For this review, take the finished solid that the model builds, in its own axes (mm). Face numbers are marked on the shaded views. A direction names the side the tool comes from. Coordinates: 2 decimals unless noted, no trailing zeros. Loops run counter-clockwise (first coordinate to the right, second up) from the corner with the lowest first, then second, coordinate; pieces in that order, holes last. Notation, with made-up numbers: (25, -26.5) -> (52, -26.5) arc R7 cw to (52, -19.5) -> close; hole circle Ø9 at (53, -19). An arc over 180 degrees is marked (long way). Use a Markdown table: item, result.
from build123d import *

# Parameters (mm, degrees)
EXTRUDE_1_DEPTH     = 30
SKETCH_3_R          = 9.25
CUT_EXTRUDE_1_DEPTH = 30
SKETCH_4_R          = 2.75
CUT_EXTRUDE_2_DEPTH = 30
CHAMFER_1_SIZE      = 5


with BuildPart() as part:
    # 草图1 → 凸台-拉伸1 (new body)
    with BuildSketch(Plane.XY):
        with BuildLine():
            Line((0, 0), (40, 0))
            ThreePointArc((40, 0), (43.535533906, -1.464466094), (45, -5))
            Line((45, -5), (45, -55))
            Line((45, -55), (41, -55))
            Line((41, -55), (41, -5))
            ThreePointArc((41, -5), (40.707106781, -4.292893219), (40, -4))
            Line((40, -4), (0, -4))
            Line((0, -4), (0, 0))
        make_face()
    extrude(amount=EXTRUDE_1_DEPTH)

    # 草图3 → 切除-拉伸1 (cut)
    with BuildSketch(Plane(origin=(45, 0, 0), x_dir=(0, 0, -1), z_dir=(1, 0, 0))):
        with Locations((-15, -40)):
            Circle(SKETCH_3_R)
    extrude(amount=-CUT_EXTRUDE_1_DEPTH, mode=Mode.SUBTRACT)

    # 草图4 → 切除-拉伸2 (cut)
    with BuildSketch(Plane(origin=(0, 0, 0), x_dir=(1, 0, 0), z_dir=(0, 1, 0))):
        with Locations(Location((5, -5, 0), (0, 0, 180))):
            Circle(SKETCH_4_R)
        with Locations(Location((25, -25, 0), (0, 0, 180))):
            Circle(SKETCH_4_R)
    extrude(amount=-CUT_EXTRUDE_2_DEPTH, mode=Mode.SUBTRACT)

    # 倒角1
    chamfer_1_edges = [part.edges().sort_by_distance(p)[0] for p in [
        (43, -55, 0),
        (0, -2, 30),
        (43, -55, 30),
        (0, -2, 0),
    ]]
    chamfer(chamfer_1_edges, length=CHAMFER_1_SIZE)


solid = part.part
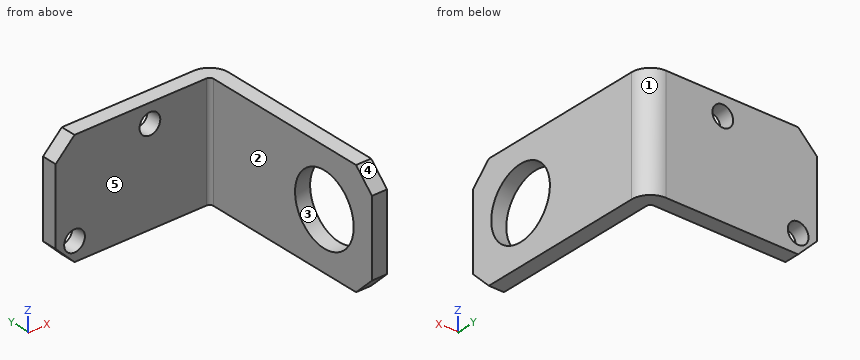
(1) Mouldability with a two-part tool opening along Y and no side actions: class the marked faces 1, 2 and 3 as pulls with the +Y half, pulls with the -Y half, needs draft (parallel to the pull), parting line crosses it, or undercut.
Found:
| item | result |
|---|---|
| face 1 | pulls with the +Y half |
| face 2 | needs draft |
| face 3 | undercut |
(2) Take a section at D-D on z = 25.75. Write out the cut boundary in (x, y).
Found:
| item | result |
|---|---|
| outline | (0.75, -4) -> (22.35, -4) -> (22.35, 0) -> (0.75, 0) -> close; (27.65, -4) -> (40, -4) arc R1 cw to (41, -5) -> (41, -54.25) -> (45, -54.25) -> (45, -5) arc R5 ccw to (40, 0) -> (27.65, 0) -> close |
(3) For the marked faces 4 and 5, list the 3-axis set-ups (+Z, -Z, +X, -X, +Y, -Y) from which the entire face can be reached by the end or side of a thin tool; tool diameter is ignored.
Found:
| item | result |
|---|---|
| face 4 | +Z, +X, -X, -Y |
| face 5 | +Z, -Z, -X, -Y |
(4) Take a section at B-B on x = 25. Write out the cut boundary in (y, z), plus the area to 3 significant figures.
Found:
| item | result |
|---|---|
| outline | (-4, 0) -> (0, 0) -> (0, 22.25) -> (-4, 22.25) -> close; (-4, 27.75) -> (0, 27.75) -> (0, 30) -> (-4, 30) -> close |
| area | 98.0 mm^2 |
(5) Take a section at C-C on y = -40. Write out the cut boundary in (x, z), plus the area to 3 significant figures.
Found:
| item | result |
|---|---|
| outline | (41, 0) -> (45, 0) -> (45, 5.75) -> (41, 5.75) -> close; (41, 24.25) -> (45, 24.25) -> (45, 30) -> (41, 30) -> close |
| area | 46.0 mm^2 |
(6) For line 1 along Z through (x, y) = (25, -1); line 2 along Z through (x, y) = (5, -1.55); line 3 along Y through (x, z) = (14.5, 8), list the stretches that pass through material, from the lowest coordinate up.
Found:
| item | result |
|---|---|
| line 1 | z = 0 to 22.25, 27.75 to 30 |
| line 2 | z = 0 to 2.25, 7.75 to 30 |
| line 3 | y = -4 to 0 |
(7) For pin 1 Ø12 at (y, z) = (-20.5, 16) entering from -X; pin 2 Ø11 at (y, z) = (-40, 15) entering from +X; pin 3 Ø7 at (x, z) = (5, 5) entering from +Y; pin 4 Ø5 at (x, z) = (31, 13) entering from -Y, all flat-tipped, find the tip position at first contact; note any pin that passes through.
Found:
| item | result |
|---|---|
| pin 1 | stops at x = 41 |
| pin 2 | passes through |
| pin 3 | stops at y = 0 |
| pin 4 | stops at y = -4 |
(8) Take a section at A-A on z = 15. Write out the cut boundary in (x, y), plus the area to 3 significant figures.
Found:
| item | result |
|---|---|
| outline | (0, -4) -> (40, -4) arc R1 cw to (41, -5) -> (41, -30.75) -> (45, -30.75) -> (45, -5) arc R5 ccw to (40, 0) -> (0, 0) -> close; (41, -55) -> (45, -55) -> (45, -49.25) -> (41, -49.25) -> close |
| area | 305 mm^2 |
